```python
from build123d import *

# Parameters (mm, degrees)
SKETCH_1_W          = 200
SKETCH_1_H          = 310
EXTRUDE_1_DEPTH     = 5
SKETCH_2_W          = 150
SKETCH_2_H          = 250
CUT_EXTRUDE_1_DEPTH = 185.729532019
FILLET_1_R          = 3
SKETCH_13_W         = 170
SKETCH_13_H         = 280
CUT_EXTRUDE_2_DEPTH = 5
HOLE_WIZARD_M5_4_D  = 4.2
FILLET_2_R          = 5
HOLE_WIZARD_M5_5_D  = 4.2
HOLE_WIZARD_M5_6_D  = 4.2


with BuildPart() as part:
    # 草图1 → 凸台-拉伸1 (new, symmetric)
    with BuildSketch(Plane(origin=(0, 0, 0), x_dir=(1, 0, 0), z_dir=(0, 1, 0))):
        Rectangle(SKETCH_1_W, SKETCH_1_H)
    extrude(amount=EXTRUDE_1_DEPTH, both=True)

    # 草图2 → 切除-拉伸1 (cut, through all)
    with BuildSketch(Plane.XZ.offset(5)):
        Rectangle(SKETCH_2_W, SKETCH_2_H)
    extrude(amount=-CUT_EXTRUDE_1_DEPTH, mode=Mode.SUBTRACT)

    # 圆角1
    fillet_1_edges = [part.edges().sort_by_distance(p)[0] for p in [
        (75, 0, 125),
        (75, 0, -125),
        (-75, 0, -125),
        (-75, 0, 125),
    ]]
    fillet(fillet_1_edges, radius=FILLET_1_R)

    # 草图13 → 切除-拉伸2 (cut)
    with BuildSketch(Plane.XZ.offset(5)):
        Rectangle(SKETCH_13_W, SKETCH_13_H)
    extrude(amount=-CUT_EXTRUDE_2_DEPTH, mode=Mode.SUBTRACT)

    # M5 螺纹孔4 (through all)
    with Locations(Plane(origin=(0, 5, 0), x_dir=(1, 0, 0), z_dir=(0, 1, 0))):
        with Locations((92.5, 105), (92.5, 125), (-92.5, 105), (-92.5, 125)):
            Hole(HOLE_WIZARD_M5_4_D / 2)

    # 圆角2
    fillet_2_edges = [part.edges().sort_by_distance(p)[0] for p in [
        (85, -2.5, 140),
        (85, -2.5, -140),
        (-85, -2.5, -140),
        (-85, -2.5, 140),
    ]]
    fillet(fillet_2_edges, radius=FILLET_2_R)

    # M5 螺纹孔5 (through all)
    with Locations(Plane(origin=(0, 5, 0), x_dir=(1, 0, 0), z_dir=(0, 1, 0))):
        with Locations((-90, -103.5), (-90, -143.5), (90, -103.5), (90, -143.5)):
            Hole(HOLE_WIZARD_M5_5_D / 2)

    # M5 螺纹孔6 (through all)
    with Locations(Plane(origin=(0, 0, 0), x_dir=(-1, 0, 0), z_dir=(0, -1, 0))):
        with Locations((75, -130), (-75, -130), (75, 130), (-75, 130)):
            Hole(HOLE_WIZARD_M5_6_D / 2)


solid = part.part
```
Input: part model. Units: mm. Frame: model coordinates. Give positions to 0.01 mm unless a question says otherwise; leave off trailing zeros. Order: outer loops, then holes, each group sorted by start corner. A loop starts at its lowest first (then second) coordinate and runs counter-clockwise, first axis right, second up. Notation, with made-up numbers: (55.25, 13) - (84.25, 13) arc R14 ccw to (84.25, 27) - close; hole circle Ø6 at (46.25, -38.5). An arc over 180 degrees is marked (long way). Use a Markdown table: item, result.
(1) Section query B-B (y = -3.5). State how many separate pieces and enclosed holes the cut face has, then the cut area to 3 significant figures.
Computed values:
| item | result |
|---|---|
| separate pieces | 1 |
| enclosed holes | 9 |
| area | 14,300 mm2 |
(2) Draft query along Z for faces 1 (the flat face through (-1, 0, 155)), 2 (the flat face through (-76, 0, 11)), 3 (the flat face through (100, 0, 2)). Return one class per face: released by +Z, released by -Z, zero draft, split by the parting line, or undercut.
Computed values:
| item | result |
|---|---|
| face 1 | released by +Z |
| face 2 | undercut |
| face 3 | zero draft |
(3) Line query: line 1 (X direction, y = 2.55, z = 130); line 2 (Z direction, x = -92.5, y = 2.5); line 3 (X direction, y = -2.75, z = 143.5). Output: solid intervals per line, ascending. Write a range as from..to.
Computed values:
| item | result |
|---|---|
| line 1 | x = -100..-77.1, -72.9..72.9, 77.1..100 |
| line 2 | z = -155..-127.1, -122.9..-107.1, -102.9..155 |
| line 3 | x = -100..-92.1, -87.9..87.9, 92.1..100 |
(4) Pin query (flat end, axial travel): pin 1 (2.5 mm diameter, centred on x = 90, z = 103.5, fed in from -Y); pin 2 (6.5 mm diameter, centred on x = 75, z = 130, fed in from -Y). Return the tip coordinate at first contact, or that it passes through.
Computed values:
| item | result |
|---|---|
| pin 1 | passes through |
| pin 2 | stops at y = 0 |
(5) Section query A-A (x = -56). Output: boundary loops of the cut face in (y, z), then the cut area to 3 significant figures.
Computed values:
| item | result |
|---|---|
| outline | (-5, -155) - (5, -155) - (5, -125) - (0, -125) - (0, -140) - (-5, -140) - close; (-5, 140) - (0, 140) - (0, 125) - (5, 125) - (5, 155) - (-5, 155) - close |
| area | 450 mm2 |
